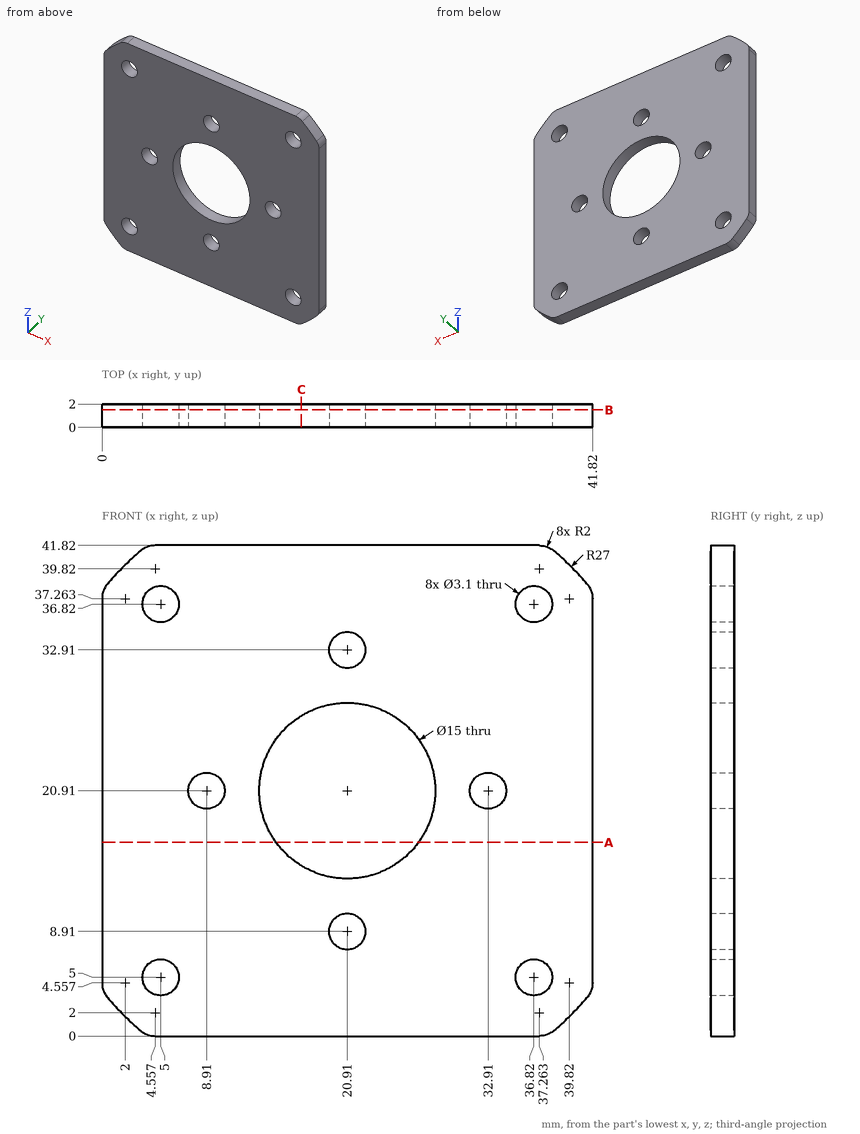
Answer from the drawing. Dimensions are ordinates in mm from the lowest x, y and z of the part. Round coordinates to 2 decimals unless told otherwise and drop trailing zeros. Loops run counter-clockwise (first coordinate to the right, second up) from the corner with the lowest first, then second, coordinate; pieces in that order, holes last.
(1) The part is cut by section A-A, the plane z = 16.5. Give the vertices of the cut face in (x, y).
Computed values:
outline: (0, 0) - (14.84, 0) - (14.84, 2) - (0, 2) - close; (26.98, 0) - (41.82, 0) - (41.82, 2) - (26.98, 2) - close
(2) The part is cut by section B-B, the plane y = 1.5. Give the number of separate pieces and of enclosed holes in the cut face, and give its area (3 significant figures).
Computed values:
separate pieces: 1
enclosed holes: 9
area: 1,480 mm2
(3) Find the intervals of material crossed by L1, parallel to Z at x = 21, y = 0.9; L2, parallel to Z at x = 20, y = 1.1 (1 decimal); L3, parallel to X at y = 1.65, z = 36 (1 decimal), in increasing order.
Computed values:
L1: z = 0 to 7.36, 10.46 to 13.41, 28.41 to 31.36, 34.46 to 41.82
L2: z = 0 to 7.7, 10.2 to 13.5, 28.4 to 31.7, 34.2 to 41.8
L3: x = 0 to 3.7, 6.3 to 35.5, 38.1 to 41.8
(4) This flat-tipped pin is pushed along its axis until it touches: P1, Ø2.5, axis at x = 8.91, z = 20.91, coming from the +Y side. Where does it stop, or does it pass through?
Computed values:
P1: passes through
(5) The part is cut by section C-C, the plane x = 17. Give the vertices of the cut face in (y, z).
Computed values:
outline: (0, 0) - (2, 0) - (2, 14.51) - (0, 14.51) - close; (0, 27.31) - (2, 27.31) - (2, 41.82) - (0, 41.82) - close
